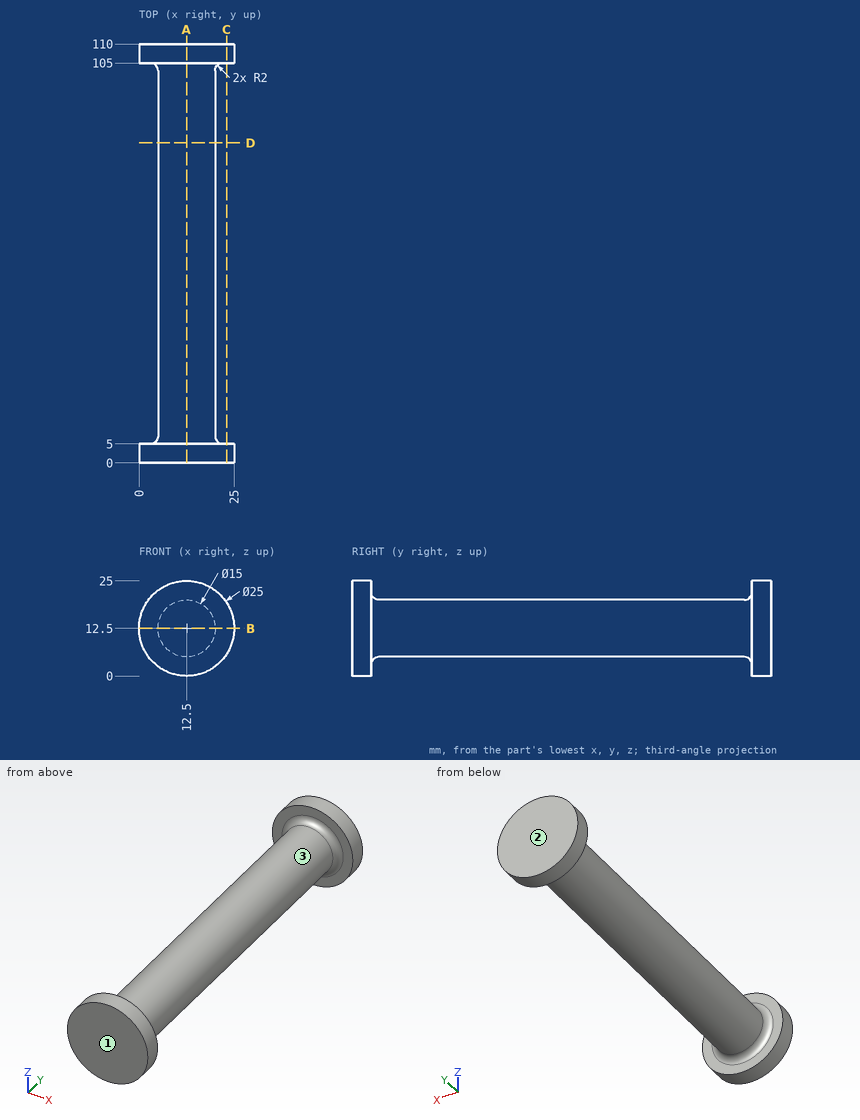
Design review of the part shown in the three views and the two pictorial views. Dimensions are in mm from the part's minimum x, y and z. Round coordinates to 2 decimals unless told otherwise and drop trailing zeros. Order: outer loops, then holes, each group sorted by start corner. A loop starts at its lowest first (then second) coordinate and runs counter-clockwise, first axis right, second up. Notation, with made-up numbers: (9, 27) - (33, 27) arc R15 ccw to (33, 54) - close; hole circle Ø7 at (8.5, 88). An arc over 180 degrees is marked (long way). Answer in a Markdown table with one row per item.
(1) Mouldability with a two-part tool opening along Y and no side actions: class the marked faces 1, 2 and 3 as released by +Y, released by -Y, zero draft, split by the parting line, or undercut.
Result set:
| item | result |
|---|---|
| face 1 | released by -Y |
| face 2 | released by +Y |
| face 3 | undercut |
(2) For line 1 (Y direction, x = 11.5, z = 2.5); line 2 (Z direction, x = 13, y = 85); line 3 (X direction, y = 69, z = 18.5), list the stretches that pass through material, from the lowest coordinate up. Write a range as from..to.
Result set:
| item | result |
|---|---|
| line 1 | y = 0..5, 105..110 |
| line 2 | z = 5.02..19.98 |
| line 3 | x = 8..17 |
(3) Take a section at C-C on x = 23. Write out the cut boundary in (y, z), plus the area to 3 significant figures.
Result set:
| item | result |
|---|---|
| outline | (0, 5.72) - (5, 5.72) - (5, 19.28) - (0, 19.28) - close; (105, 5.72) - (110, 5.72) - (110, 19.28) - (105, 19.28) - close |
| area | 136 mm2 |
(4) Take a section at D-D on y = 84. Write out the cut boundary in (x, z), plus the area to 3 significant figures.
Result set:
| item | result |
|---|---|
| outline | circle Ø15 at (12.5, 12.5) |
| area | 177 mm2 |
(5) Take a section at A-A on x = 12.5. Write out the cut boundary in (y, z), plus the area to 3 significant figures.
Result set:
| item | result |
|---|---|
| outline | (0, 0) - (5, 0) - (5, 3) arc R2 cw to (7, 5) - (103, 5) arc R2 cw to (105, 3) - (105, 0) - (110, 0) - (110, 25) - (105, 25) - (105, 22) arc R2 cw to (103, 20) - (7, 20) arc R2 cw to (5, 22) - (5, 25) - (0, 25) - close |
| area | 1,750 mm2 |
(6) Clearance check with flat-ended pins moving along their axes: P1, Ø12, axis at x = 11.5, y = 14.5, coming from the +Z side; P2, Ø2, axis at x = 20, y = 60, coming from the +Z side. State where each tip first meets the part, or that it passes through.
Result set:
| item | result |
|---|---|
| P1 | stops at z = 20 |
| P2 | stops at z = 16.24 |
(7) Take a section at B-B on z = 12.5. Write out the cut boundary in (x, y), plus the area to 3 significant figures.
Result set:
| item | result |
|---|---|
| outline | (0, 0) - (25, 0) - (25, 5) - (22, 5) arc R2 cw to (20, 7) - (20, 103) arc R2 cw to (22, 105) - (25, 105) - (25, 110) - (0, 110) - (0, 105) - (3, 105) arc R2 cw to (5, 103) - (5, 7) arc R2 cw to (3, 5) - (0, 5) - close |
| area | 1,750 mm2 |
